Work out the finished part from the listing and answer in its coordinate system (mm). Give positions to 0.01 mm unless a question says otherwise; leave off trailing zeros. Loops run counter-clockwise (first coordinate to the right, second up) from the corner with the lowest first, then second, coordinate; pieces in that order, holes last. Notation, with made-up numbers: M 39,-38.5 L 52,-38.5 A13 ccw 52,-25.5 Z; hole C -22.75,63 d8. An arc over 180 degrees is marked long. Write item = value, one per line. Start each with the question number.
1. Section A-A on z = -0.5 is taken. Determine the outline of the cut face in (x, y) (3 decimals).
2. Section B-B on y = 100 is taken. Determine the outline of the cut face in (x, z), plus the area to 3 significant figures.
3. Flat-ended cylindrical pins translate along their axes: pin 1 Ø1.5 at (x, z) = (-17, 5) entering from +Y; pin 2 Ø4 at (y, z) = (140, -2) entering from +X; pin 3 Ø8 at (x, z) = (32, -2.5) entering from +Y. Find the tip coordinate at first contact, or state that the pin passes through.
4. Consider L1, parallel to X at y = 183, z = -0.5; L2, parallel to X at y = 86, z = -4.5; L3, parallel to Y at x = 23.5, z = -0.5. Determine where each line is inside the solid, lowest interval first. Write a range as [from, to].
```python
from build123d import *


with BuildPart() as part:
    # 扫描1: sweep along a path in 草图1
    with BuildLine(Plane.XY) as sweep_1_path:
        Line((133.935000245, 322.9682066), (50.990864547, -352.799410804))
        ThreePointArc((50.990864547, -352.799410804), (-34.525526627, -420.379935429), (-103.043927412, -335.613142274))
        Line((-103.043927412, -335.613142274), (-35.006384485, 341.817662407))
        ThreePointArc((-35.006384485, 341.817662407), (58.993428728, 417.799266002), (133.935000245, 322.9682066))
    # 草图2 → 扫描1 (sweep)
    with BuildSketch(Plane(origin=(0, 322.9682066, 0), x_dir=(1, 0, 0), z_dir=(0, 1, 0))):
        Polygon((133.935000245, 8.5), (133.935000245, -8.5), (117.935000245, -5), (117.935000245, 5), align=None)
    sweep(path=sweep_1_path.line)


solid = part.part
```
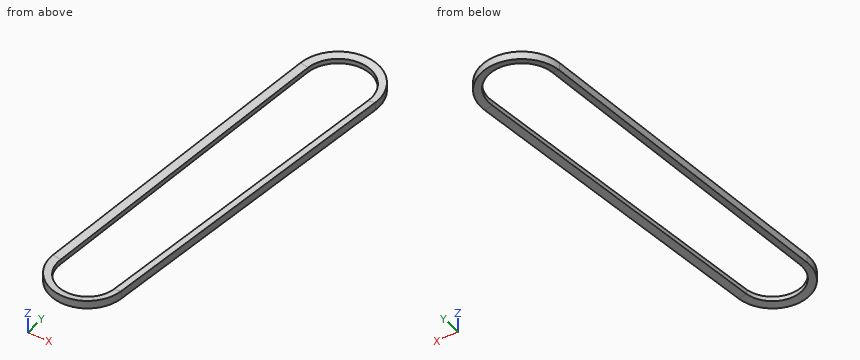
Verdict:
q1.outline = M -103.044,-335.613 A77.5 ccw 50.991,-352.799 L 133.935,322.968 A85 ccw long -35.006,341.818 Z; hole M -87.048,-335.261 A61.65 ccw 34.991,-352.799 L 117.935,322.968 A69.147 ccw long -19.01,342.17 Z
q2.outline = M -59.29,-8.5 L -43.33,-5 L -43.33,5 L -59.29,8.5 Z; M 90.57,-5 L 106.57,-8.5 L 106.57,8.5 L 90.57,5 Z
q2.area = 431 mm2
q3.pin_1 = 387.11
q3.pin_2 = 111.72
q3.pin_3 = 417.23
q4.L1 = [-50.96, -35], [100.76, 116.76]
q4.L2 = [-60.7, -44.74], [88.85, 104.85]
q4.L3 = [-403.05, -380.2], [397.37, 414.23]
